Here's how the part is built. I have some questions about the finished solid (model axes, mm). Round coordinates to 2 decimals unless told otherwise and drop trailing zeros. Order: outer loops, then holes, each group sorted by start corner. A loop starts at its lowest first (then second) coordinate and runs counter-clockwise, first axis right, second up.
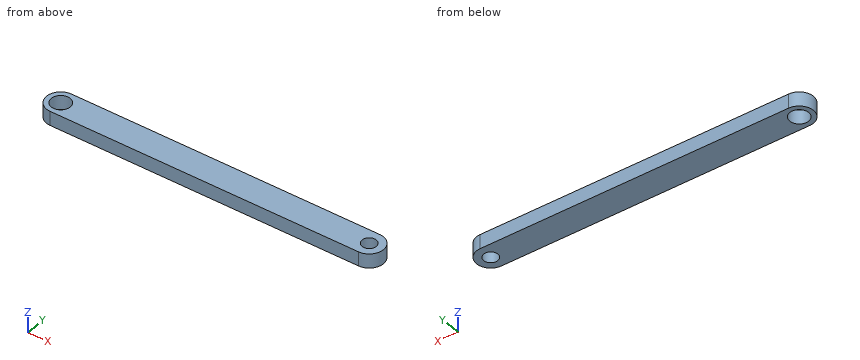
```python
from build123d import *

# Parameters (mm, degrees)
SKETCH1_R           = 4
SKETCH1_R_2         = 3
BOSS_EXTRUDE1_DEPTH = 6
SCALE1_SCALE        = 0.5


with BuildPart() as part:
    # Sketch1 → Boss-Extrude1 (new body)
    with BuildSketch(Plane.XY):
        with BuildLine():
            Line((-32.375641401, 3), (97.624358599, 3))
            ThreePointArc((97.624358599, 3), (103.624358599, -3), (97.624358599, -9))
            Line((97.624358599, -9), (-32.375641401, -9))
            ThreePointArc((-32.375641401, -9), (-38.375641401, -3), (-32.375641401, 3))
        make_face()
        with Locations((-32.375641401, -3)):
            Circle(SKETCH1_R, mode=Mode.SUBTRACT)
        with Locations((97.624358599, -3)):
            Circle(SKETCH1_R_2, mode=Mode.SUBTRACT)
    extrude(amount=BOSS_EXTRUDE1_DEPTH)


with BuildPart() as part_1:
    # Scale1: scaled about (0, 0, 0)
    add(part.part.scale(SCALE1_SCALE))


solid = part_1.part
```
1. If we section it at B-B, the plane z = 1.4: Write out the boundary of the cut face in (x, y).
Evaluation:
outline: (-16.19, -4.5) - (48.81, -4.5) arc R3 ccw to (48.81, 1.5) - (-16.19, 1.5) arc R3 ccw to start; hole circle Ø4 at (-16.19, -1.5); hole circle Ø3 at (48.81, -1.5)
2. If we section it at A-A, the plane y = -1.5: Write out the boundary of the cut face in (x, z).
Evaluation:
outline: (-19.19, 0) - (-18.19, 0) - (-18.19, 3) - (-19.19, 3) - close; (-14.19, 0) - (47.31, 0) - (47.31, 3) - (-14.19, 3) - close; (50.31, 0) - (51.81, 0) - (51.81, 3) - (50.31, 3) - close
3. I'm going to push a flat-ended pin straight in: P1, Ø2.5, axis at x = -16.19, y = -1.5, coming from the +Z side. Where does the tip first touch, or does it pass through?
Evaluation:
P1: passes through
4. I need wall thicknesses on probe 1 along X at (y, z) = (-1.9, 0.4); probe 2 along Y at (x, z) = (49, 1.25); probe 3 along X at (y, z) = (-0.7, 0.9). Which ranges of each line are inside material? Lowest first, please.
Evaluation:
probe 1: x = -19.16 to -18.15, -14.23 to 47.37, 50.26 to 51.79
probe 2: y = -4.49 to -2.99, -0.01 to 1.49
probe 3: x = -19.08 to -18.02, -14.35 to 47.54, 50.08 to 51.7
